Here's how the part is built. I have some questions about the finished solid (model axes, mm). A direction names the side the tool comes from. Round coordinates to 2 decimals unless told otherwise and drop trailing zeros. Write each loop counter-clockwise with the first axis right and the second up, starting at its lowest first coordinate (ties: lowest second). Pieces come first, ordered by that corner, then holes. Notation, with made-up numbers: M -32,53.5 L -11,53.5 A21 cw -11,68.5 Z; hole C -10,8 d11. An arc over 180 degrees is marked long. Use one line per item in the form item = value. Start each with the question number.
Q1. I want a section at A-A on x = 8. List the corners of the cut face in (y, z) for me, and give its area (4 significant figures).
Q2. We'd pull the mould along X, two halves only. Please class faces 4 (the face through (4.75, 2.28, 0.05)), 5 (the face through (-4, 0.1, 3)), 6 (the face through (29, -1, 0)), 7 (the face through (3, 2, 8)): +X half, -X half, draft (parallel to the pull), parting line (faces both ways), or undercut.
Q3. For faces 1 (the face through (-16, 2, 6)), 2 (the face through (26, -7.5, 0)), 3 (the face through (2, 0.4, -6.1)), which set-ups out of +Z, -Z, +X, -X, +Y, -Y let a thin tool reach every point of the face, with its end or its side?
Q4. I'm going to push flat-ended pins straight in: pin 1 Ø5 at (x, z) = (-14.5, 1) entering from -Y; pin 2 Ø4 at (y, z) = (-2.5, -0.5) entering from -X; pin 3 Ø3 at (x, z) = (-2.5, -5) entering from -Y. Where does each tip first touch, or does it pass through?
Q5. I want a section at C-C on z = 4. List the corners of the cut face in (x, y) for me, and give its area (3 significant figures).
Q6. I need wall thicknesses on line 1 along Z through (x, y) = (9, 1.5); line 2 along Y through (x, z) = (26.1, 0); line 3 along X through (y, z) = (0.5, -5.75). Which ranges of each line are inside material? Lowest first, please. Write a range as from..to.
Q7. I want a section at B-B on y = -3.5. List the corners of the cut face in (x, z) for me, and give its area (3 significant figures).
Q8. I want a section at D-D on x = 24. List the corners of the cut face in (y, z) for me.
```python
from build123d import *

# Parameters (mm, degrees)
SKETCH1_W             = 46
SKETCH1_H             = 16
BOSS_EXTRUDE1_DEPTH   = 4.5
SKETCH2_W             = 16
SKETCH2_H             = 12
BOSS_EXTRUDE2_DEPTH   = 6
SKETCH3_R             = 1
CUT_EXTRUDE1_DEPTH    = 10
M3_TAPPED_HOLE1_D     = 2.5
M3_TAPPED_HOLE1_DEPTH = 7.5
M3_TAPPED_HOLE1_TIP   = 0.751075774
CHAMFER1_SIZE         = 2
CUT_EXTRUDE2_DEPTH    = 7.5
CUT_EXTRUDE3_DEPTH    = 2.75
FILLET1_R             = 3
FILLET2_R             = 2
CUT_EXTRUDE4_DEPTH    = 15
CUT_EXTRUDE5_DEPTH    = 15
CHAMFER2_SIZE         = 0.5


with BuildPart() as part:
    # Sketch1 → Boss-Extrude1 (new body)
    with BuildSketch(Plane(origin=(0, 0, 0), x_dir=(1, 0, 0), z_dir=(0, 1, 0))):
        Rectangle(SKETCH1_W, SKETCH1_H)
    extrude(amount=BOSS_EXTRUDE1_DEPTH)

    # Sketch2 → Boss-Extrude2 (add)
    with BuildSketch(Plane(origin=(23, 0, 0), x_dir=(0, 0, -1), z_dir=(1, 0, 0))):
        with Locations((0, -1.5)):
            Rectangle(SKETCH2_W, SKETCH2_H)
    extrude(amount=BOSS_EXTRUDE2_DEPTH)

    # Sketch3 → Cut-Extrude1 (cut)
    with BuildSketch(Plane(origin=(29, 0, 0), x_dir=(0, 0, -1), z_dir=(1, 0, 0))):
        with Locations((0, -3.5)):
            Circle(SKETCH3_R)
    extrude(amount=-CUT_EXTRUDE1_DEPTH, mode=Mode.SUBTRACT)

    # M3 Tapped Hole1
    with Locations(Plane(origin=(29, -3.5, 0), x_dir=(0, 0, 1), z_dir=(1, 0, 0))):
        with Locations((0, 0)):
            Hole(M3_TAPPED_HOLE1_D / 2, depth=M3_TAPPED_HOLE1_DEPTH)
            with Locations((0, 0, -(M3_TAPPED_HOLE1_DEPTH + M3_TAPPED_HOLE1_TIP / 2))):  # 118° drill point
                Cone(0, M3_TAPPED_HOLE1_D / 2, M3_TAPPED_HOLE1_TIP, mode=Mode.SUBTRACT)

    # Chamfer1
    chamfer1_edges = [part.edges().sort_by_distance(p)[0] for p in [
        (26, -7.5, -8),
        (26, -7.5, 8),
    ]]
    chamfer(chamfer1_edges, length=CHAMFER1_SIZE)

    # Sketch5 → Cut-Extrude2 (cut, symmetric)
    with BuildSketch(Plane.ZY.offset(5.5)):
        Polygon((-1.4, 0), (-15.004762523, 0), (-15.004762523, 2.891781544), align=None)
    extrude(amount=CUT_EXTRUDE2_DEPTH, both=True, mode=Mode.SUBTRACT)

    # Sketch6 → Cut-Extrude3 (cut, symmetric)
    with BuildSketch(Plane.ZY.offset(4)):
        Polygon((-1.389489576, 0.1), (-8, 1.505107367), (-8, -0.5), (8, -0.5), (8, 0.1), align=None)
    extrude(amount=CUT_EXTRUDE3_DEPTH, both=True, mode=Mode.SUBTRACT)

    # Fillet1
    fillet1_edges = [part.edges().sort_by_distance(p)[0] for p in [
        (-4, 1.505107367, -8),
    ]]
    fillet(fillet1_edges, radius=FILLET1_R)

    # Fillet2
    fillet2_edges = [part.edges().sort_by_distance(p)[0] for p in [
        (-4, 0.1, -1.389489576),
    ]]
    fillet(fillet2_edges, radius=FILLET2_R)

    # Sketch7 → Cut-Extrude4 (cut)
    with BuildSketch(Plane(origin=(0, 4.5, 0), x_dir=(1, 0, 0), z_dir=(0, 1, 0))):
        with BuildLine():
            Line((-18.5, -2), (-13.5, -2))
            ThreePointArc((-13.5, -2), (-11.5, -4), (-13.5, -6))
            Line((-13.5, -6), (-18.5, -6))
            ThreePointArc((-18.5, -6), (-20.5, -4), (-18.5, -2))
        make_face()
    extrude(amount=-CUT_EXTRUDE4_DEPTH, mode=Mode.SUBTRACT)

    # Sketch8 → Cut-Extrude5 (cut)
    with BuildSketch(Plane(origin=(0, 4.5, 0), x_dir=(1, 0, 0), z_dir=(0, 1, 0))):
        with BuildLine():
            Line((7, 2.25), (13, 2.25))
            ThreePointArc((13, 2.25), (15.25, 0), (13, -2.25))
            Line((13, -2.25), (7, -2.25))
            ThreePointArc((7, -2.25), (4.75, 0), (7, 2.25))
        make_face()
    extrude(amount=-CUT_EXTRUDE5_DEPTH, mode=Mode.SUBTRACT)

    # Chamfer2
    chamfer2_edges = [part.edges().sort_by_distance(p)[0] for p in [
        (-1.25, 2.668666387, -8),
        (-6.75, 2.668666387, -8),
    ]]
    chamfer(chamfer2_edges, length=CHAMFER2_SIZE)


solid = part.part
```
Reported:
q1.outline = M 0,-8 L 4.5,-8 L 4.5,-2.25 L 0,-2.25 Z; M 0,2.25 L 4.5,2.25 L 4.5,8 L 0,8 Z
q1.area = 51.75 mm^2
q2.face_4 = undercut
q2.face_5 = undercut
q2.face_6 = +X half
q2.face_7 = draft
q3.face_1 = +Y, -Y
q3.face_2 = +Z, -Z, +X, -X, -Y
q3.face_3 = -Z, -Y
q4.pin_1 = 0
q4.pin_2 = 23
q4.pin_3 = 0.55
q5.outline = M -23,0 L -20.5,0 L -20.5,4.5 L -23,4.5 Z; M -11.5,0 L -6.75,0 L -6.75,0.1 L -1.25,0.1 L -1.25,0 L 23,0 L 23,-7.5 L 29,-7.5 L 29,4.5 L -11.5,4.5 Z
q5.area = 238 mm^2
q6.line_1 = -8..-2.25, 2.25..8
q6.line_2 = -7.5..-4.75, -2.25..4.5
q6.line_3 = -23..-13, 2..29
q7.outline = M 23,-8 L 29,-8 L 29,-1.25 L 23,-1.25 Z; M 23,1.25 L 29,1.25 L 29,8 L 23,8 Z
q7.area = 81.0 mm^2
q8.outline = M -7.5,-6 L -5.5,-8 L 4.5,-8 L 4.5,8 L -5.5,8 L -7.5,6 Z; hole C -3.5,0 d2.5
